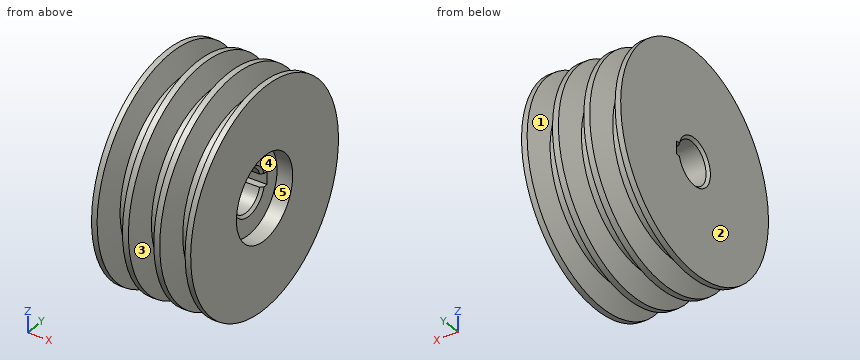
```python
from build123d import *

# Parameters (mm, degrees)
PATTERN_LINEAR_1_COUNT = 3
PATTERN_LINEAR_1_PITCH = 12
CHAMFER_1_SIZE         = 1
SKETCH_4_W             = 5
SKETCH_4_H             = 2.700657875
CUT_EXTRUDE_1_DEPTH    = 71.512410255


with BuildPart() as part:
    # 草图1 → 旋转1 (revolve)
    with BuildSketch(Plane.XY, mode=Mode.PRIVATE) as revolve_1_sk:
        Polygon((0, 8), (0, 42), (38, 42), (38, 16), (32, 16), (32, 8), align=None)
    revolve(revolve_1_sk.sketch.rotate(Axis((0, 0, 0), (1, 0, 0)), 90), axis=Axis((0, 0, 0), (1, 0, 0)))

    # 草图2 → 切除-旋转1 (revolve, cut)
    with BuildSketch(Plane.XY, mode=Mode.PRIVATE) as cut_revolve_1_sk:
        Polygon((9.10988523, 33), (11.861461363, 42), (2.138538637, 42), (4.89011477, 33), align=None)
    cut_revolve_1 = revolve(cut_revolve_1_sk.sketch.rotate(Axis((0, 0, 0), (1, 0, 0)), 90), axis=Axis((0, 0, 0), (1, 0, 0)), mode=Mode.SUBTRACT)

    # 阵列(线性)1: 切除-旋转1 ×3
    with Locations(*[(i * PATTERN_LINEAR_1_PITCH, 0, 0) for i in range(1, PATTERN_LINEAR_1_COUNT)]):
        add(cut_revolve_1, mode=Mode.SUBTRACT)

    # 倒角1
    chamfer_1_edges = [part.edges().sort_by_distance(p)[0] for p in [
        (32, 0, -8),
        (0, 0, -8),
    ]]
    chamfer(chamfer_1_edges, length=CHAMFER_1_SIZE)

    # 草图4 → 切除-拉伸1 (cut, through all)
    with BuildSketch(Plane.ZY):
        with Locations((0, 8.949671014)):
            Rectangle(SKETCH_4_W, SKETCH_4_H)
    extrude(amount=-CUT_EXTRUDE_1_DEPTH, mode=Mode.SUBTRACT)


solid = part.part
```
The model under review builds one solid part; all positions refer to its coordinate system, in mm. Face numbers are marked on the shaded views. A direction names the side the tool comes from. Round coordinates to 2 decimals unless told otherwise and drop trailing zeros. Write each loop counter-clockwise with the first axis right and the second up, starting at its lowest first coordinate (ties: lowest second). Pieces come first, ordered by that corner, then holes. Notation, with made-up numbers: (55.5, 20) - (59.5, 20) arc R25 cw to (59.5, 43) - close; hole circle Ø3 at (84, 18). An arc over 180 degrees is marked (long way). Answer as CSV lines item,"result". Start each with the question number.
(1) We need section B-B on y = 35. Give the number of separate pieces and of enclosed holes in the cut face, plus the area to 3 significant figures.
(2) Draft analysis for pull direction X (two halves, no side actions). For the marked faces 3, 4 and 5, state which applies: pulls with the +X half, pulls with the -X half, needs draft (parallel to the pull), parting line crosses it, or undercut.
(3) We need section C-C on x = 27.5. State the section outline as (y, z) points, plus the area to 3 significant figures.
(4) For pin 1 Ø1.5 at (x, z) = (14, 0) entering from -Y; pin 2 Ø5 at (x, z) = (14.5, -32) entering from -Y; pin 3 Ø3 at (x, y) = (19.5, 9.5) entering from -Z, all flat-tipped, find the tip position at first contact; note any pin that passes through.
(5) To check wall thickness, follow line 1 (X direction, y = -35.5, z = 14); line 2 (Y direction, x = 12.5, z = 0); line 3 (Y direction, x = 20.25, z = 0). State the ranges of each line that lie inside material, in increasing order.
(6) For the marked faces 1 and 2, list the 3-axis set-ups (+Z, -Z, +X, -X, +Y, -Y) from which the entire face can be reached by the end or side of a thin tool; tool diameter is ignored.
(7) We need section A-A on x = 18. State the section outline as (y, z) points.
Worked answers:
1,separate pieces,"4"
1,enclosed holes,"0"
1,area,"800 mm²"
2,face 3,"undercut"
2,face 4,"pulls with the +X half"
2,face 5,"needs draft"
3,outline,"circle Ø75.09 at (0, 0); hole (7.6, -2.5) - (10.3, -2.5) - (10.3, 2.5) - (7.6, 2.5) arc R8 ccw (long way) to start"
3,area,"4,220 mm²"
4,pin 1,"y = -42"
4,pin 2,"y = -29.87"
4,pin 3,"z = -32.02"
5,line 1,"0 to 3.31, 10.69 to 15.31, 22.69 to 27.31, 34.69 to 38"
5,line 2,"-42 to -8, 10.3 to 42"
5,line 3,"-33 to -8, 10.3 to 33"
6,face 1,"none"
6,face 2,"+Z, -Z, -X, +Y, -Y"
7,outline,"circle Ø66 at (0, 0); hole (7.6, -2.5) - (10.3, -2.5) - (10.3, 2.5) - (7.6, 2.5) arc R8 ccw (long way) to start"
